from build123d import *

# Parameters (mm, degrees)
SKETCH2_R          = 23
CUT_EXTRUDE1_DEPTH = 17
SKETCH3_R          = 16
CUT_EXTRUDE2_DEPTH = 606.281099986
CHAMFER1_SIZE      = 2
CUT_EXTRUDE3_DEPTH = 20
CUT_EXTRUDE4_DEPTH = 13
CIRPATTERN1_COUNT  = 6


with BuildPart() as part:
    # Sketch1 → Revolve1 (revolve)
    with BuildSketch(Plane(origin=(0, 318.5, 0), x_dir=(-1, 0, 0), z_dir=(0, -1, 0)), mode=Mode.PRIVATE) as revolve1_sk:
        Polygon((176, 77.5), (176, 87.5), (30, 87.5), (26, 174.5), (0, 174.5), (0, 26.1), (227, 26.1), (227, 53.1), (222, 53.1), (222, 50.1), (219, 50.1), (219, 51.1), (199, 51.1), (199, 50.1), (196, 50.1), (196, 51.1), (196, 77.5), align=None)
    revolve(revolve1_sk.sketch.rotate(Axis((0, 318.5, 0), (0, 0, -1)), 180), axis=Axis((0, 318.5, 0), (0, 0, -1)))

    # Sketch2 → Cut-Extrude1 (cut)
    with BuildSketch(Plane.XY.offset(-26.1)):
        with Locations((0, 318.5)):
            Circle(SKETCH2_R)
    extrude(amount=-CUT_EXTRUDE1_DEPTH, mode=Mode.SUBTRACT)

    # Sketch3 → Cut-Extrude2 (cut, through all)
    with BuildSketch(Plane.XY.offset(-43.1)):
        with Locations((0, 318.5)):
            Circle(SKETCH3_R)
    extrude(amount=-CUT_EXTRUDE2_DEPTH, mode=Mode.SUBTRACT)

    # Chamfer1
    chamfer1_edges = [part.edges().sort_by_distance(p)[0] for p in [
        (-23, 318.5, -26.1),
    ]]
    chamfer(chamfer1_edges, length=CHAMFER1_SIZE)

    # Sketch4 → Cut-Extrude3 (cut)
    with BuildSketch(Plane.XY.offset(-26.1)):
        with BuildLine():
            Line((-8, 606.712422614), (-8, 408.5))
            ThreePointArc((-8, 408.5), (0, 400.5), (8, 408.5))
            Line((8, 408.5), (8, 606.712422614))
            Line((8, 606.712422614), (-8, 606.712422614))
        make_face()
    cut_extrude3 = extrude(amount=-CUT_EXTRUDE3_DEPTH, mode=Mode.SUBTRACT)

    # Sketch5 → Cut-Extrude4 (cut)
    with BuildSketch(Plane.XY.offset(-33.1)):
        with BuildLine():
            Line((-15, 626.113520772), (-15, 408.5))
            ThreePointArc((-15, 408.5), (0, 393.5), (15, 408.5))
            Line((15, 408.5), (15, 626.113520772))
            Line((15, 626.113520772), (-15, 626.113520772))
        make_face()
    cut_extrude4 = extrude(amount=-CUT_EXTRUDE4_DEPTH, mode=Mode.SUBTRACT)

    # CirPattern1: Cut-Extrude3, Cut-Extrude4 ×6 about axis
    cirpattern1_axis = Axis((0, 318.5, 0), (0, 0, 1))
    add([cut_extrude3.rotate(cirpattern1_axis, i * 360 / CIRPATTERN1_COUNT) for i in range(1, CIRPATTERN1_COUNT)], mode=Mode.SUBTRACT)
    add([cut_extrude4.rotate(cirpattern1_axis, i * 360 / CIRPATTERN1_COUNT) for i in range(1, CIRPATTERN1_COUNT)], mode=Mode.SUBTRACT)


solid = part.part
Could you check a few things on this model? Use its own coordinates, in mm. A direction names the side the tool comes from. Give positions to 0.01 mm unless a question says otherwise; leave off trailing zeros. Loops run counter-clockwise (first coordinate to the right, second up) from the corner with the lowest first, then second, coordinate; pieces in that order, holes last. Notation, with made-up numbers: (83, -40) -> (100, -40) arc R19 cw to (100, -13) -> close; hole circle Ø4 at (56.5, 29). An arc over 180 degrees is marked (long way). Answer as CSV lines item,"result". Start each with the question number.
(1) Which directions (+Z, -Z, +X, -X, +Y, -Y) give clear straight access to the entire face, cutting with the end or side of a thin tool? Please do faces 1 (the flat face through (0, 471, -46.1)), 2 (the flat face through (-128.723, 410.139, -39.509)), 3 (the flat face through (5, 334, -43.1)).
(2) We'd pull the mould along Y, two halves only. Please class faces 4 (the flat face through (10, 470, -33.1)), 5 (the flat face through (143.723, 384.158, -39.509)), 6 (the conical face through (12.907, 343.316, -131.609)): released by +Y, released by -Y, zero draft, split by the parting line, or undercut.
(3) I need wall thicknesses on probe 1 along Y at (x, z) = (0, -50.35); probe 2 along Y at (x, z) = (26.5, -51); probe 3 along X at (y, z) = (318, -37). Which ranges of each line are inside material? Lowest first, please.
(4) If we section it at D-D on z = -139.5: Write out the boundary of the cut face in (x, y).
(5) I'm going to push flat-ended pins straight in: pin 1 Ø4 at (y, z) = (158, -76) entering from +X; pin 2 Ø9 at (x, y) = (-6, 131) entering from -Z; pin 3 Ø8 at (y, z) = (441.5, -62.5) entering from +X. Where does each tip first touch, or does it pass through?
(6) If we section it at B-B on z = -69: Write out the boundary of the cut face in (x, y), then the cut area to 3 significant figures.
Computed:
1,face 1,"+Y"
1,face 2,"none"
1,face 3,"+Z"
2,face 4,"zero draft"
2,face 5,"undercut"
2,face 6,"split by the parting line"
3,probe 1,"y = 91.5 to 96.5, 99.5 to 119.5, 122.5 to 302.5, 334.5 to 514.5, 517.5 to 537.5, 540.5 to 545.5"
3,probe 2,"y = 93.05 to 98.09, 101.11 to 121.27, 124.3 to 512.7, 515.73 to 535.89, 538.91 to 543.95"
3,probe 3,"x = -227 to -22.99, 22.99 to 227"
4,outline,"circle Ø55.22 at (0, 318.5); hole circle Ø32 at (0, 318.5)"
5,pin 1,"stops at x = 115.3"
5,pin 2,"stops at z = -77.5"
5,pin 3,"stops at x = 155.74"
6,outline,"circle Ø392 at (0, 318.5); hole circle Ø32 at (0, 318.5)"
6,area,"120,000 mm2"
